CAD build for the part. Positions are in the model's coordinates, mm. Face numbers are marked on the shaded views. Give positions to 0.01 mm unless a question says otherwise; leave off trailing zeros. Order: outer loops, then holes, each group sorted by start corner. A loop starts at its lowest first (then second) coordinate and runs counter-clockwise, first axis right, second up.
Item 1: Band-saw the part on C-C on z = 3.25. Give the cut face in (x, y).
Item 2: Wall check: L1, parallel to Y at x = 0, z = 14.5; L2, parallel to X at y = 19, z = 8.5; L3, parallel to X at y = 23.5, z = 28.25. Give the ranges that are in metal, low to high.
Item 3: Flat gauge pins, fed straight in: P1, Ø10, axis at x = -32, z = 20.5, coming from the +Y side; P2, Ø10, axis at x = 11, z = 26.5, coming from the -Y side; P3, Ø12, axis at x = -3.5, z = 22.5, coming from the +Y side. Where does each tip first touch, or does it go through?
Item 4: Band-saw the part on A-A on y = 0. Give the cut face in (x, z), plus the area to 3 significant figures.
Item 5: Band-saw the part on D-D on z = 26.5. Give the cut face in (x, y).
Item 6: Two-plate mould, pull along Y, no slides. Class the marked faces 1, 2 and 3: released by +Y, released by -Y, zero draft, split by the parting line, or undercut.
```python
from build123d import *

# Parameters (mm, degrees)
SKETCH1_R           = 60
SKETCH1_R_2         = 27.5
BOSS_EXTRUDE1_DEPTH = 30
CHAMFER1_SIZE       = 5
CHAMFER2_SIZE       = 2


with BuildPart() as part:
    # Sketch1 → Boss-Extrude1 (new body)
    with BuildSketch(Plane.XY):
        Circle(SKETCH1_R)
        Circle(SKETCH1_R_2, mode=Mode.SUBTRACT)
    extrude(amount=BOSS_EXTRUDE1_DEPTH)

    # Chamfer1
    chamfer1_edges = [part.edges().sort_by_distance(p)[0] for p in [
        (-60, 0, 0),
        (-60, 0, 30),
    ]]
    chamfer(chamfer1_edges, length=CHAMFER1_SIZE)

    # Chamfer2
    chamfer2_edges = [part.edges().sort_by_distance(p)[0] for p in [
        (-27.5, 0, 30),
    ]]
    chamfer(chamfer2_edges, length=CHAMFER2_SIZE)


solid = part.part
```
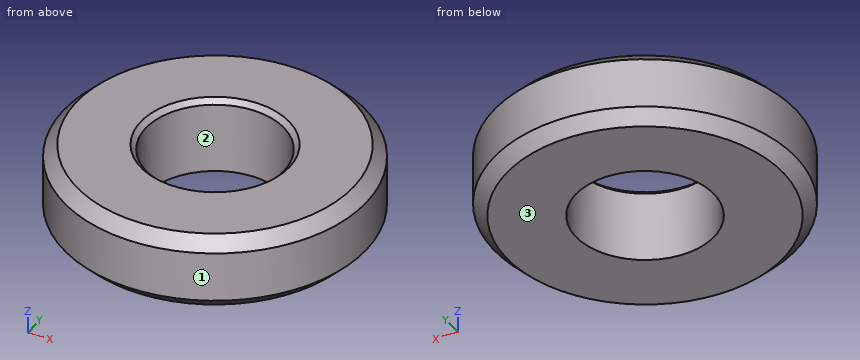
The answers:
1. outline: circle Ø116.5 at (0, 0); hole circle Ø55 at (0, 0)
2. L1: y = -60 to -27.5, 27.5 to 60
2. L2: x = -56.91 to -19.88, 19.88 to 56.91
2. L3: x = -51.66 to -14.76, 14.76 to 51.66
3. P1: stops at y = 53.58
3. P2: stops at y = -59.68
3. P3: stops at y = 60
4. outline: (-60, 5) - (-55, 0) - (-27.5, 0) - (-27.5, 28) - (-29.5, 30) - (-55, 30) - (-60, 25) - close; (27.5, 0) - (55, 0) - (60, 5) - (60, 25) - (55, 30) - (29.5, 30) - (27.5, 28) - close
4. area: 1,900 mm2
5. outline: circle Ø117 at (0, 0); hole circle Ø55 at (0, 0)
6. face 1: split by the parting line
6. face 2: undercut
6. face 3: zero draft
